Input: part model. Units: mm. Frame: model coordinates. A direction names the side the tool comes from. Give positions to 0.01 mm unless a question says otherwise; leave off trailing zeros. Loops run counter-clockwise (first coordinate to the right, second up) from the corner with the lowest first, then second, coordinate; pieces in that order, holes last. Notation, with made-up numbers: (-28.75, 61) -> (-14.75, 61) arc R13 cw to (-14.75, 73) -> close; hole circle Ø3 at (88, -9). An arc over 180 degrees is marked (long way). Answer in a Markdown table with one row per item. Add a question column.
```python
from build123d import *

# Parameters (mm, degrees)
BASE_PLATE_DEPTH             = 4
FLANGE_RISER_SKETCH_W        = 65.921827793
FLANGE_RISER_SKETCH_H        = 4
FLANGE_RISER_DEPTH           = 10
CURVED_FLANGE_DEPTH          = 66
PLATE_CORNER_FILLETS_R10_R   = 10
PLATE_CORNER_CHAMFER_18_SIZE = 18
MOUNTING_HOLES_SKETCH_R      = 5
MOUNTING_HOLES_2X_DEPTH      = 66


with BuildPart() as part:
    # Base Plate Sketch → Base Plate (new body)
    with BuildSketch(Plane(origin=(0, 0, 0), x_dir=(1, 0, 0), z_dir=(0, 1, 0))):
        Polygon((-54, -32), (54, -32), (54, -5.811207063), (0, 32), (-54, 32), align=None)
    extrude(amount=BASE_PLATE_DEPTH)

    # Flange Riser Sketch → Flange Riser (add)
    with BuildSketch(Plane(origin=(15.035081933, 0, -21.472322293), x_dir=(-0.8191520442889909, 0, -0.5735764363510474), z_dir=(0.5735764363510474, 0, -0.8191520442889909))):
        with Locations((-14.606467934, 2)):
            Rectangle(FLANGE_RISER_SKETCH_W, FLANGE_RISER_SKETCH_H)
    extrude(amount=FLANGE_RISER_DEPTH)

    # Curved Flange Profile Sketch → Curved Flange (add)
    with BuildSketch(Plane(origin=(38.964918067, 0, 27.283529357), x_dir=(0.5735764363510477, 0, -0.8191520442889908), z_dir=(0.8191520442889907, 0, 0.5735764363510476))):
        with BuildLine():
            Line((23.720397301, 4), (33.088147536, 4))
            ThreePointArc((33.088147536, 4), (40.61496291, 6.654035613), (44.812372275, 13.442158279))
            Line((44.812372275, 13.442158279), (47.116411582, 24.003044212))
            Line((47.116411582, 24.003044212), (51.162040745, 23.120420475))
            Line((51.162040745, 23.120420475), (48.17789207, 9.442158279))
            ThreePointArc((48.17789207, 9.442158279), (43.980482705, 2.654035613), (36.453667331, 0))
            Line((36.453667331, 0), (24.245794341, 0))
            Line((24.245794341, 0), (23.720397301, 4))
        make_face()
    extrude(amount=-CURVED_FLANGE_DEPTH)

    # Plate Corner Fillets R10
    plate_corner_fillets_r10_edges = [part.edges().sort_by_distance(p)[0] for p in [
        (-54, 2, -32),
        (54, 2, 32),
    ]]
    fillet(plate_corner_fillets_r10_edges, radius=PLATE_CORNER_FILLETS_R10_R)

    # Plate Corner Chamfer 18
    plate_corner_chamfer_18_edges = [part.edges().sort_by_distance(p)[0] for p in [
        (-54, 2, 32),
    ]]
    chamfer(plate_corner_chamfer_18_edges, length=PLATE_CORNER_CHAMFER_18_SIZE)

    # Mounting Holes Sketch → Mounting Holes 2x (cut)
    with BuildSketch(Plane(origin=(0, 4, 0), x_dir=(1, 0, 0), z_dir=(0, 1, 0))):
        with Locations(Location((-44, 22, 0), (0, 0, 270))):
            Circle(MOUNTING_HOLES_SKETCH_R)
        with Locations(Location((44, -22, 0), (0, 0, 270))):
            Circle(MOUNTING_HOLES_SKETCH_R)
    extrude(amount=-MOUNTING_HOLES_2X_DEPTH, mode=Mode.SUBTRACT)


solid = part.part
```
1) Material intervals for line 1 along Y through (x, z) = (-16, 26); line 2 along X through (y, z) = (1.65, 22); line 3 along X through (y, z) = (2.65, -22), sorted ascending.
2) Section A-A on x = -41. Output: boundary loops of the cut face in (y, z), and give its area (3 significant figures).
3) Section B-B on y = 20.25. Output: boundary loops of the cut face in (x, z).
4) Reachability of faces 1 (the face through (-4, 4, 7)), 2 (the face through (-22, 2, -32)), 3 (the face through (54, 2, 14)), 4 (the face through (37.59, 2.73, -27.48)), 5 (the face through (3, 2, 32)) from +Z, -Z, +X, -X, +Y, -Y: full face, straight path, thin tool, end or side. Return the list, or none.
5) Pull-direction query (X, two-part tool) for faces 6 (the face through (48.957, 2.028, 21.349)), 7 (the face through (40.48, 23.568, -31.609)), 8 (the face through (35.556, 6.583, -24.576)), 9 (the face through (-39.043, 2.028, -22.651)); classes: +X half, -X half, draft (parallel to the pull), parting line (faces both ways), or undercut.
6) Pin query (flat end, axial travel): pin 1 (12 mm diameter, centred on y = 17, z = -36, fed in from -X); pin 2 (12 mm diameter, centred on x = -24, z = -36, fed in from +Y); pin 3 (3 mm diameter, centred on y = 1, z = 16, fed in from +X); pin 4 (6 mm diameter, centred on x = 44, z = 22, fed in from -Y). Return the tip coordinate at first contact, or that it passes through.
Working result:
| question | item | result |
|---|---|---|
| 1 | line 1 | y = 0 to 4 |
| 1 | line 2 | x = -46 to 39, 49 to 54 |
| 1 | line 3 | x = -54 to -49, -39 to 45.25 |
| 2 | outline | (0, -32) -> (4, -32) -> (4, -26) -> (0, -26) -> close; (0, -18) -> (4, -18) -> (4, 27) -> (0, 27) -> close |
| 2 | area | 204 mm2 |
| 3 | outline | (11.46, -48.5) -> (13.89, -51.97) -> (67.95, -14.11) -> (65.52, -10.64) -> close |
| 4 | face 1 | +Z, -X, +Y |
| 4 | face 2 | -Z, -X, +Y, -Y |
| 4 | face 3 | +Z, +X, +Y, -Y |
| 4 | face 4 | -Z, +X, -Y |
| 4 | face 5 | +Z, +X, -X, +Y, -Y |
| 5 | face 6 | undercut |
| 5 | face 7 | +X half |
| 5 | face 8 | -X half |
| 5 | face 9 | undercut |
| 6 | pin 1 | stops at x = 19.2 |
| 6 | pin 2 | stops at y = 4 |
| 6 | pin 3 | stops at x = 54 |
| 6 | pin 4 | passes through |
